Work out the finished part from the listing and answer in its coordinate system (mm). A direction names the side the tool comes from. Coordinates: 2 decimals unless noted, no trailing zeros. Order: outer loops, then holes, each group sorted by start corner. A loop starts at its lowest first (then second) coordinate and runs counter-clockwise, first axis right, second up.
1. Flat-ended cylindrical pins translate along their axes: pin 1 Ø10 at (x, z) = (15.5, 61) entering from +Y; pin 2 Ø2 at (x, z) = (-12, 136.5) entering from -Y; pin 3 Ø12 at (y, z) = (22, 89.5) entering from +X. Find the tip coordinate at first contact, or state that the pin passes through.
2. Find the intervals of material crossed by probe 1 along Y at (x, z) = (0.5, 19); probe 2 along Z at (x, y) = (19, 13); probe 3 along X at (y, z) = (2.5, 14.5), in increasing order.
3. Determine the mould class of faces 4 (the cylindrical face through (25.865, -10.724, 65.592)), 5 (the cylindrical face through (-2.4, -4.5, 142.7)), 6 (the flat face through (-7, 19, 58)) for opening direction Y: +Y half, -Y half, draft (parallel to the pull), parting line (faces both ways), or undercut.
4. The part is cut by section B-B, the plane z = 113.5. Give the vertices of the cut face in (x, y).
5. The part is cut by section A-A, the plane z = 138.5. Give the vertices of the cut face in (x, y), then the cut area to 3 significant figures.
6. A tool of negligible diameter and unlimited length cuts with its end or side. For faces 1 (the flat face through (-4, 4, 0)), 2 (the flat face through (-7, 19, 78.4)), 3 (the cylindrical face through (19.98, -0.88, 29.1)), from which of +Z, -Z, +X, -X, +Y, -Y can it reach the whole face along a straight path? Write none if from no direction.
```python
from build123d import *

# Parameters (mm, degrees)
SKETCH_1_R              = 20
EXTRUDE_1_DEPTH         = 58
SKETCH_2_R              = 28
EXTRUDE_2_DEPTH         = 20.4
SKETCH_3_R              = 20
EXTRUDE_3_DEPTH         = 79.1
CHAMFER_1_SIZE          = 5
CHAMFER_2_SIZE          = 1
HOLE_WIZARD_M12_1_D     = 10.2
HOLE_WIZARD_M12_1_DEPTH = 29.25
HOLE_WIZARD_M12_1_TIP   = 3.064389157
HOLE_WIZARD_M12_2_D     = 10.2
HOLE_WIZARD_M12_2_DEPTH = 29.25
HOLE_WIZARD_M12_2_TIP   = 3.064389157


with BuildPart() as part:
    # 草图1 → 凸台-拉伸1 (new body)
    with BuildSketch(Plane.XY):
        with Locations(Location((0, 0, 0), (0, 0, 180))):
            Circle(SKETCH_1_R)
    extrude(amount=EXTRUDE_1_DEPTH)

    # 草图2 → 凸台-拉伸2 (add)
    with BuildSketch(Plane.XY.offset(58)):
        Circle(SKETCH_2_R)
    extrude(amount=EXTRUDE_2_DEPTH)

    # 草图3 → 凸台-拉伸3 (add)
    with BuildSketch(Plane.XY.offset(78.4)):
        with Locations(Location((0, 0, 0), (0, 0, 180))):
            Circle(SKETCH_3_R)
    extrude(amount=EXTRUDE_3_DEPTH)

    # 倒角1
    chamfer_1_edges = [part.edges().sort_by_distance(p)[0] for p in [
        (-28, 0, 78.4),
    ]]
    chamfer(chamfer_1_edges, length=CHAMFER_1_SIZE)

    # 倒角2
    chamfer_2_edges = [part.edges().sort_by_distance(p)[0] for p in [
        (20, 0, 157.5),
        (20, 0, 0),
    ]]
    chamfer(chamfer_2_edges, length=CHAMFER_2_SIZE)

    # M12 螺纹孔1
    with Locations(Plane(origin=(0, 0, 0), x_dir=(-1, 0, 0), z_dir=(0, 0, -1))):
        with Locations((0, 0)):
            Hole(HOLE_WIZARD_M12_1_D / 2, depth=HOLE_WIZARD_M12_1_DEPTH)
            with Locations((0, 0, -(HOLE_WIZARD_M12_1_DEPTH + HOLE_WIZARD_M12_1_TIP / 2))):  # 118° drill point
                Cone(0, HOLE_WIZARD_M12_1_D / 2, HOLE_WIZARD_M12_1_TIP, mode=Mode.SUBTRACT)

    # M12 螺纹孔2
    with Locations(Plane.XY.offset(157.5)):
        with Locations((0, 0)):
            Hole(HOLE_WIZARD_M12_2_D / 2, depth=HOLE_WIZARD_M12_2_DEPTH)
            with Locations((0, 0, -(HOLE_WIZARD_M12_2_DEPTH + HOLE_WIZARD_M12_2_TIP / 2))):  # 118° drill point
                Cone(0, HOLE_WIZARD_M12_2_D / 2, HOLE_WIZARD_M12_2_TIP, mode=Mode.SUBTRACT)


solid = part.part
```
Geometry says:
1. pin 1: stops at y = 25.96
1. pin 2: stops at y = -16.7
1. pin 3: stops at x = 12
2. probe 1: y = -19.99 to -5.08, 5.08 to 19.99
2. probe 2: z = 58 to 78.38
2. probe 3: x = -19.84 to -4.45, 4.45 to 19.84
3. face 4: parting line
3. face 5: undercut
3. face 6: draft
4. outline: circle Ø40 at (0, 0)
5. outline: circle Ø40 at (0, 0); hole circle Ø10.2 at (0, 0)
5. area: 1,170 mm2
6. face 1: -Z, +X, -X, +Y, -Y
6. face 2: +Z
6. face 3: -Z
